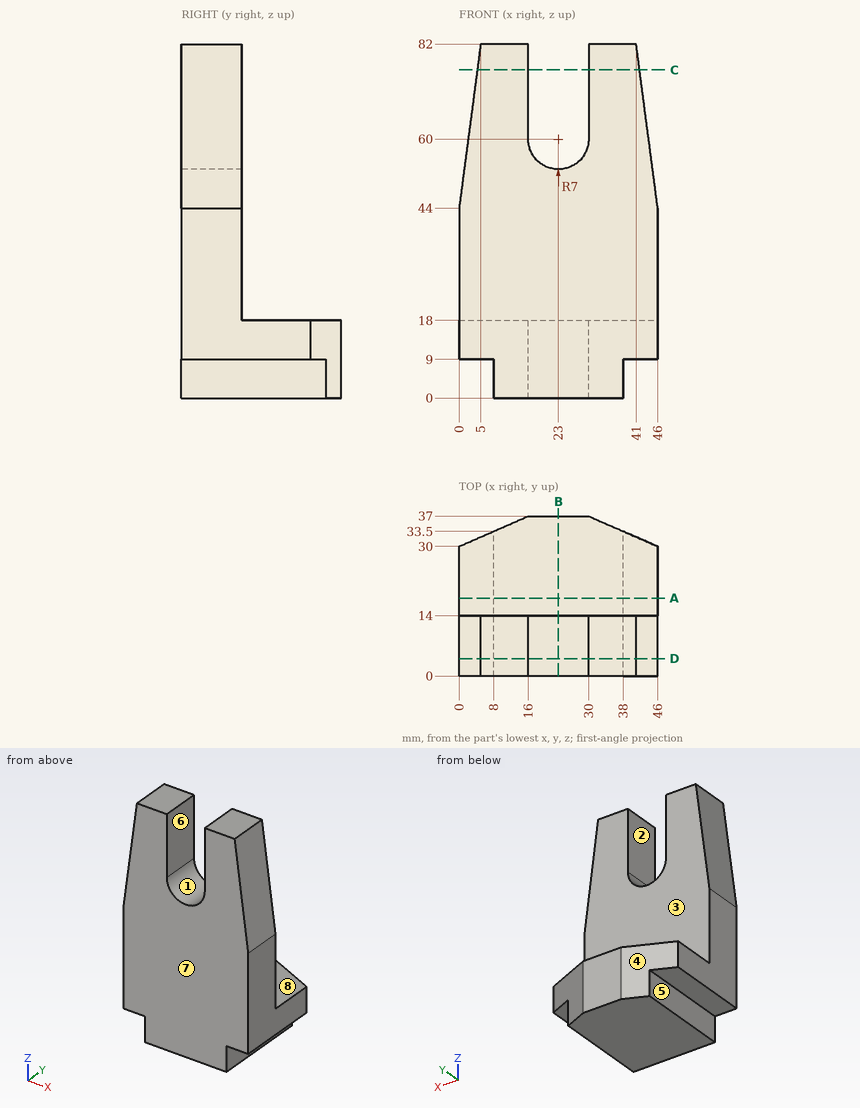
Here's the drawing with two shaded views (mm, measured from the low corner). I have some questions. A direction names the side the tool comes from. Coordinates: 2 decimals unless noted, no trailing zeros. Loops run counter-clockwise (first coordinate to the right, second up) from the corner with the lowest first, then second, coordinate; pieces in that order, holes last. Notation, with made-up numbers: M 2,-31.5 L 6,-31.5 A28 cw 6,-1.5 Z; hole C 25,61 d3. An arc over 180 degrees is marked long. Put each result on its own line as item: value. Start each with the question number.
(1) I need wall thicknesses on probe 1 along Z at (x, y) = (5.5, 32); probe 2 along Y at (x, z) = (16, 21.5); probe 3 along Z at (x, y) = (14, 29.5). Which ranges of each line are inside material? Lowest first, please.
(2) We'd pull the mould along X, two halves only. Please class the marked faces 1, 2, 3 and 4: +X half, -X half, draft (parallel to the pull), parting line (faces both ways), or undercut.
(3) Imagine slicing it at D-D on y = 4. List the corners of the cut face in (x, z) for me.
(4) Imagine slicing it at C-C on z = 76. List the corners of the cut face in (x, y) for me, and give its area (3 significant figures).
(5) Will these pins go through, and if not, where does the flat tip stop? pin 1 Ø4.5 at (y, z) = (24, 5.5) entering from +X; pin 2 Ø6.5 at (x, y) = (42.5, 13.5) entering from -Z; pin 3 Ø4.5 at (y, z) = (8.5, 4) entering from -X.
(6) Imagine slicing it at A-A on y = 18. List the corners of the cut face in (x, z) for me.
(7) Imagine slicing it at B-B on x = 23. List the corners of the cut face in (y, z) for me, and give its area (3 significant figures).
(8) Which directions (+Z, -Z, +X, -X, +Y, -Y) give clear straight access to the entire face, cutting with the end or side of a thin tool? Please do the marked faces 5, 6, 7 and 8.
Worked answers:
1. probe 1: z = 9 to 18
1. probe 2: y = 0 to 14
1. probe 3: z = 0 to 18
2. face 1: undercut
2. face 2: undercut
2. face 3: draft
2. face 4: -X half
3. outline: M 0,9 L 8,9 L 8,0 L 38,0 L 38,9 L 46,9 L 46,44 L 41,82 L 30,82 L 30,60 A7 cw 16,60 L 16,82 L 5,82 L 0,44 Z
4. outline: M 4.21,0 L 16,0 L 16,14 L 4.21,14 Z; M 30,0 L 41.79,0 L 41.79,14 L 30,14 Z
4. area: 330 mm2
5. pin 1: stops at x = 38
5. pin 2: stops at z = 9
5. pin 3: stops at x = 8
6. outline: M 0,9 L 8,9 L 8,0 L 38,0 L 38,9 L 46,9 L 46,18 L 0,18 Z
7. outline: M 0,0 L 37,0 L 37,18 L 14,18 L 14,53 L 0,53 Z
7. area: 1,160 mm2
8. face 5: -Z, -X, +Y, -Y
8. face 6: +Z, +Y, -Y
8. face 7: +Z, -Z, +X, -X, -Y
8. face 8: +Z, +X, -X, +Y
